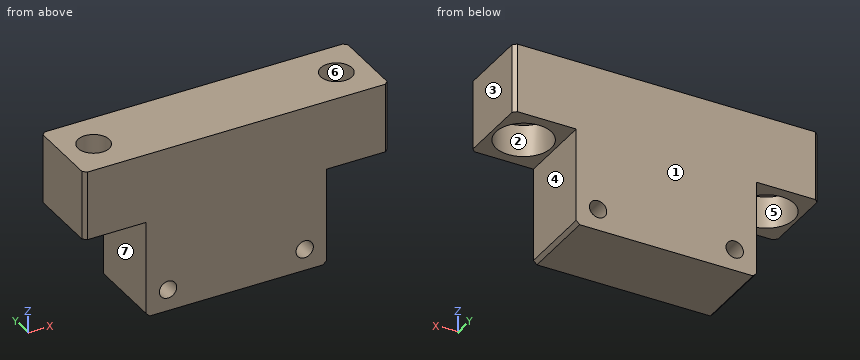
```python
from build123d import *

# Parameters (mm, degrees)
SKETCH1_W                                            = 44
SKETCH1_H                                            = 11
BOSS_EXTRUDE1_DEPTH                                  = 24
SKETCH2_W                                            = 9
SKETCH2_H                                            = 14
CUT_EXTRUDE1_DEPTH                                   = 35.365680555
CBORE_FOR_M4_HEXAGON_SOCKET_HEAD_CAP_SCR_D           = 4.5
CBORE_FOR_M4_HEXAGON_SOCKET_HEAD_CAP_SCR_CBORE_D     = 8
CBORE_FOR_M4_HEXAGON_SOCKET_HEAD_CAP_SCR_CBORE_DEPTH = 4.6
M3_TAPPED_HOLE1_D                                    = 2.5
CHAMFER1_SIZE                                        = 0.5
CHAMFER2_SIZE                                        = 0.5


with BuildPart() as part:
    # Sketch1 → Boss-Extrude1 (new body)
    with BuildSketch(Plane.XY):
        Rectangle(SKETCH1_W, SKETCH1_H)
    extrude(amount=BOSS_EXTRUDE1_DEPTH)

    # Sketch2 → Cut-Extrude1 (cut, through all)
    with BuildSketch(Plane(origin=(0, 5.5, 0), x_dir=(1, 0, 0), z_dir=(0, 1, 0))):
        with Locations((-17.5, -7)):
            Rectangle(SKETCH2_W, SKETCH2_H)
        with Locations((17.5, -7)):
            Rectangle(SKETCH2_W, SKETCH2_H)
    extrude(amount=-CUT_EXTRUDE1_DEPTH, mode=Mode.SUBTRACT)

    # CBORE for M4 Hexagon socket head cap screws1 (through all)
    with Locations(Plane(origin=(0, 0, 14), x_dir=(-1, 0, 0), z_dir=(0, 0, -1))):
        with Locations((-17.5, 0), (17.5, 0)):
            CounterBoreHole(CBORE_FOR_M4_HEXAGON_SOCKET_HEAD_CAP_SCR_D / 2, CBORE_FOR_M4_HEXAGON_SOCKET_HEAD_CAP_SCR_CBORE_D / 2, CBORE_FOR_M4_HEXAGON_SOCKET_HEAD_CAP_SCR_CBORE_DEPTH)

    # M3 Tapped Hole1 (through all)
    with Locations(Plane(origin=(0, 5.5, 0), x_dir=(1, 0, 0), z_dir=(0, 1, 0))):
        with Locations((9.85, -3.1), (-9.85, -3.1)):
            Hole(M3_TAPPED_HOLE1_D / 2)

    # Chamfer1
    chamfer1_edges = [part.edges().sort_by_distance(p)[0] for p in [
        (22, -5.5, 19),
        (-22, -5.5, 19),
        (-22, 5.5, 19),
        (22, 5.5, 19),
    ]]
    chamfer(chamfer1_edges, length=CHAMFER1_SIZE)

    # Chamfer2
    chamfer2_edges = [part.edges().sort_by_distance(p)[0] for p in [
        (-13, 0, 0),
        (13, 0, 0),
    ]]
    chamfer(chamfer2_edges, length=CHAMFER2_SIZE)


solid = part.part
```
Could you check a few things on this model? Use its own coordinates, in mm. Face numbers are marked on the shaded views. A direction names the side the tool comes from. Round coordinates to 2 decimals unless told otherwise and drop trailing zeros. Order: outer loops, then holes, each group sorted by start corner. A loop starts at its lowest first (then second) coordinate and runs counter-clockwise, first axis right, second up. Notation, with made-up numbers: (49.5, -15.75) -> (87.5, -15.75) arc R22 ccw to (87.5, 14.25) -> close; hole circle Ø3 at (-32, 14). An arc over 180 degrees is marked (long way). One line per question, with ' | ' between items.
Q1. If we section it at A-A on y = 0: Write out the boundary of the cut face in (x, z), plus the area to 3 significant figures.
Computed values:
outline: (-22, 14) -> (-21.5, 14) -> (-21.5, 18.6) -> (-19.75, 18.6) -> (-19.75, 24) -> (-22, 24) -> close; (-15.25, 18.6) -> (-13.5, 18.6) -> (-13.5, 14) -> (-13, 14) -> (-13, 0.5) -> (-12.5, 0) -> (12.5, 0) -> (13, 0.5) -> (13, 14) -> (13.5, 14) -> (13.5, 18.6) -> (15.25, 18.6) -> (15.25, 24) -> (-15.25, 24) -> close; (19.75, 18.6) -> (21.5, 18.6) -> (21.5, 14) -> (22, 14) -> (22, 24) -> (19.75, 24) -> close; hole circle Ø2.5 at (-9.85, 3.1); hole circle Ø2.5 at (9.85, 3.1) | area: 672 mm²
Q2. If we section it at D-D on z = 3.1: Write out the boundary of the cut face in (x, y), plus the area to 3 significant figures.
Computed values:
outline: (-13, -5.5) -> (-11.1, -5.5) -> (-11.1, 5.5) -> (-13, 5.5) -> close; (-8.6, -5.5) -> (8.6, -5.5) -> (8.6, 5.5) -> (-8.6, 5.5) -> close; (11.1, -5.5) -> (13, -5.5) -> (13, 5.5) -> (11.1, 5.5) -> close | area: 231 mm²
Q3. We'd pull the mould along Y, two halves only. Please class the marked faces 1, 2 and 3: released by +Y, released by -Y, zero draft, split by the parting line, or undercut.
Computed values:
face 1: released by +Y | face 2: undercut | face 3: zero draft
Q4. If we section it at B-B on z = 22: Write out the boundary of the cut face in (x, y), plus the area to 3 significant figures.
Computed values:
outline: (-22, -5) -> (-21.5, -5.5) -> (21.5, -5.5) -> (22, -5) -> (22, 5) -> (21.5, 5.5) -> (-21.5, 5.5) -> (-22, 5) -> close; hole circle Ø4.5 at (-17.5, 0); hole circle Ø4.5 at (17.5, 0) | area: 452 mm²
Q5. If I drill on line 1 (Z direction, x = -9.85, y = 2.25); line 2 (Y direction, x = -17.5, z = 15.4); line 3 (Y direction, x = 17.5, z = 19.9), over which ranges is the centre line in solid material (lowest first)? Write a range as from..to.
Computed values:
line 1: 0..1.85, 4.35..24 | line 2: -5.5..-4, 4..5.5 | line 3: -5.5..-2.25, 2.25..5.5
Q6. Which directions (+Z, -Z, +X, -X, +Y, -Y) give clear straight access to the entire face, cutting with the end or side of a thin tool? Please do the marked faces 4, 5, 6 and 7.
Computed values:
face 4: -Z, +X, +Y, -Y | face 5: -Z | face 6: +Z, -Z | face 7: -Z, -X, +Y, -Y
Q7. I'm going to push flat-ended pins straight in: pin 1 (3.5 mm diameter, centred on y = -2, z = 7.5, fed in from +X); pin 2 (5 mm diameter, centred on x = 17.5, y = 0, fed in from +Z); pin 3 (4.5 mm diameter, centred on x = 19.5, y = -1, fed in from -Z); pin 4 (6 mm diameter, centred on x = 17.5, y = 0, fed in from -Z). Where does each tip first touch, or does it pass through?
Computed values:
pin 1: x = 13 | pin 2: z = 24 | pin 3: z = 14 | pin 4: z = 18.6
Q8. If we section it at C-C on x = 9.85: Write out the boundary of the cut face in (y, z).
Computed values:
outline: (-5.5, 0) -> (5.5, 0) -> (5.5, 1.85) -> (-5.5, 1.85) -> close; (-5.5, 4.35) -> (5.5, 4.35) -> (5.5, 24) -> (-5.5, 24) -> close
